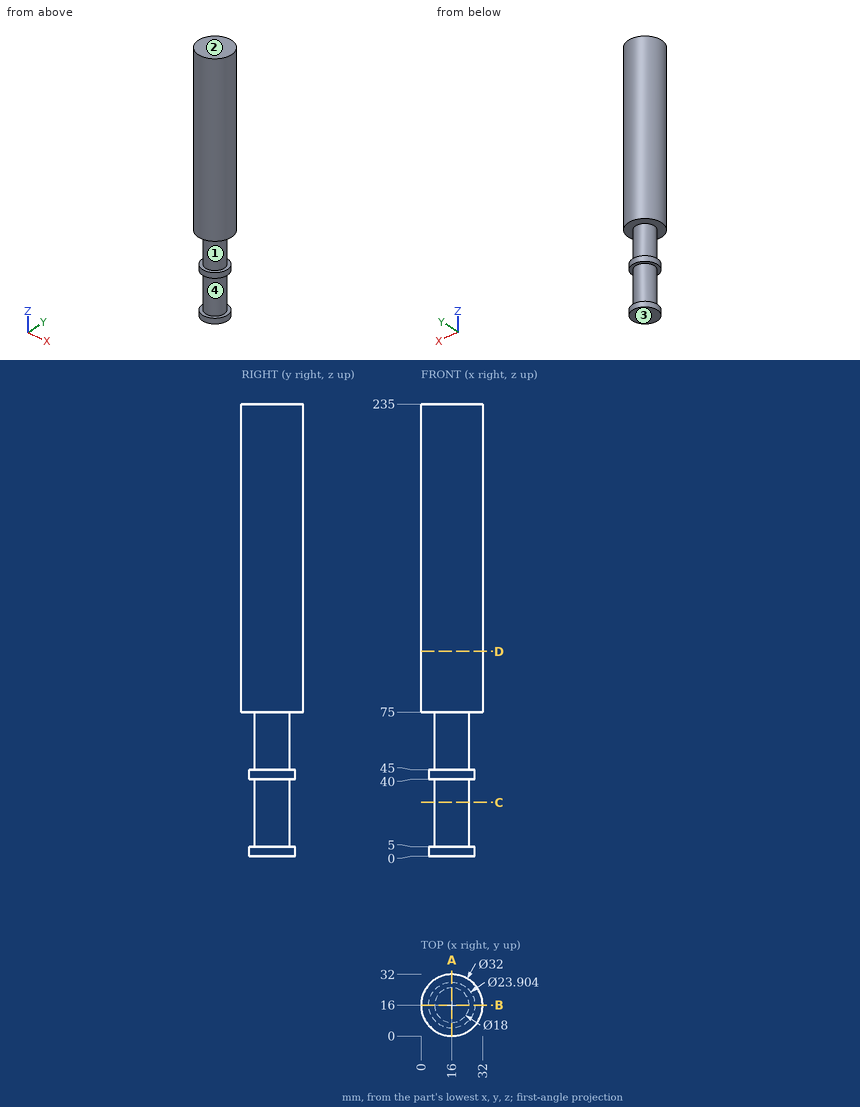
Geometry: see drawing. Coordinates: mm, zero at the bounding-box minimum. Coordinates: 2 decimals unless noted, no trailing zeros. Write each loop counter-clockwise with the first axis right and the second up, starting at its lowest first coordinate (ties: lowest second). Pieces come first, ordered by that corner, then holes.
1) Section D-D on z = 106.5. Output: boundary loops of the cut face in (x, y).
2) Section A-A on x = 16. Output: boundary loops of the cut face in (y, z), and give its area (3 significant figures).
3) Section C-C on z = 28. Output: boundary loops of the cut face in (x, y).
4) Material intervals for line 1 along Z through (x, y) = (19.5, 7.5); line 2 along Y through (x, z) = (15, 132); line 3 along Z through (x, y) = (2.5, 11.5), sorted ascending.
5) Mould query, pull axis Z, two halves, no side actions, for the marked faces 1, 2, 3 and 4. Classes: pulls with the +Z half, pulls with the -Z half, needs draft (parallel to the pull), parting line crosses it, or undercut.
6) Pin query (flat end, axial travel): pin 1 Ø10 at (x, z) = (26.5, 46) entering from -Y; pin 2 Ø8 at (y, z) = (5, 135.5) entering from +X; pin 3 Ø3 at (y, z) = (27, 85) entering from +X (1 decimal). Return the tip coordinate at first contact, or that it passes through.
Check result:
1. outline: circle Ø32 at (16, 16)
2. outline: (0, 75) - (7, 75) - (7, 45) - (4.05, 45) - (4.05, 40) - (7, 40) - (7, 5) - (4.05, 5) - (4.05, 0) - (27.95, 0) - (27.95, 5) - (25, 5) - (25, 40) - (27.95, 40) - (27.95, 45) - (25, 45) - (25, 75) - (32, 75) - (32, 235) - (0, 235) - close
2. area: 6,530 mm2
3. outline: circle Ø18 at (16, 16)
4. line 1: z = 0 to 5, 40 to 45, 75 to 235
4. line 2: y = 0.03 to 31.97
4. line 3: z = 75 to 235
5. face 1: undercut
5. face 2: pulls with the +Z half
5. face 3: pulls with the -Z half
5. face 4: undercut
6. pin 1: stops at y = 5.44
6. pin 2: stops at x = 30.39
6. pin 3: stops at x = 28.9
